The listing builds one solid part. Answer for the finished solid, in the listing's coordinates (mm). Face numbers are marked on the shaded views. A direction names the side the tool comes from. Coordinates: 2 decimals unless noted, no trailing zeros. Order: outer loops, then holes, each group sorted by start corner. A loop starts at its lowest first (then second) coordinate and runs counter-clockwise, first axis right, second up. Notation, with made-up numbers: (87, 60.5) - (143, 60.5) arc R20 cw to (143, 82.5) - close; hole circle Ø10 at (-11, 73). An arc over 180 degrees is marked (long way). Use a Markdown table: item, result. Add a question column.
Item 1: For the marked faces 1, 2 and 3, determine the directions among +Z, -Z, +X, -X, +Y, -Y from which every point of the face is accessible in a straight line to the end or side of a thin tool.
Item 2: The part is cut by section B-B, the plane x = 10. Give the vertices of the cut face in (y, z), then the cut area to 3 significant figures.
Item 3: Find the intervals of material crossed by line 1 along X through (y, z) = (2.25, 5.5); line 2 along Z through (x, y) = (-37, 0.5); line 3 along Z through (x, y) = (-64.5, 0.5), in increasing order.
Item 4: The part is cut by section C-C, the plane x = -9. Give the vertices of the cut face in (y, z).
Item 5: Flat-ended cylindrical pins translate along their axes: P1, Ø3, axis at x = -31.5, z = -3, coming from the +Y side; P2, Ø0.7, axis at x = -36, y = 6.5, coming from the -Z side; P3, Ø2, axis at x = 11, y = 5, coming from the -Z side. Find the tip coordinate at first contact, or state that the pin passes through.
Item 6: The part is cut by section D-D, the plane x = -23. Give the vertices of the cut face in (y, z), then the cut area to 3 significant figures.
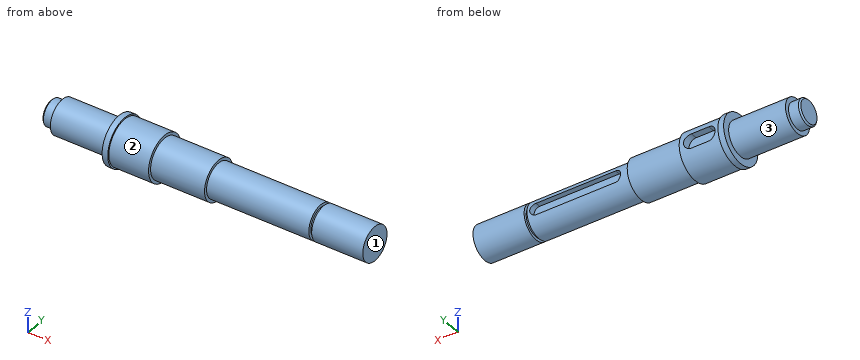
from build123d import *

# Parameters (mm, degrees)
CUT_EXTRUDE_1_DEPTH = 2.2
CUT_EXTRUDE_2_DEPTH = 2.8


with BuildPart() as part:
    # 草图1 → 旋转1 (revolve)
    with BuildSketch(Plane.XY, mode=Mode.PRIVATE) as revolve_1_sk:
        Polygon((-46.103902345, 8.5), (-44.103902345, 8.5), (-44.103902345, 8), (-30.103902345, 8), (-30.103902345, 7), (-11.103902345, 7), (-11.103902345, 6), (24.896097655, 6), (24.896097655, 5), (25.896097655, 5), (25.896097655, 6), (43.896097655, 6), (43.896097655, 0), (-70.103902345, 0), (-70.103902345, 4), (-69.603902345, 4.5), (-66.103902345, 4.5), (-66.103902345, 6), (-46.103902345, 6), align=None)
    revolve(revolve_1_sk.sketch.rotate(Axis((-70.103902345, 0, 0), (1, 0, 0)), 90), axis=Axis((-70.103902345, 0, 0), (1, 0, 0)))

    # 草图7 → 切除-拉伸1 (cut)
    with BuildSketch(Plane(origin=(0, 6, 0), x_dir=(1, 0, 0), z_dir=(0, 1, 0))):
        with BuildLine():
            Line((-6.053902345, 2), (21.946097655, 2))
            ThreePointArc((21.946097655, 2), (23.946097655, 0), (21.946097655, -2))
            Line((21.946097655, -2), (-6.053902345, -2))
            ThreePointArc((-6.053902345, -2), (-8.053902345, 0), (-6.053902345, 2))
        make_face()
    extrude(amount=-CUT_EXTRUDE_1_DEPTH, mode=Mode.SUBTRACT)

    # 草图9 → 切除-拉伸2 (cut)
    with BuildSketch(Plane(origin=(0, 8, 0), x_dir=(1, 0, 0), z_dir=(0, 1, 0))):
        with BuildLine():
            Line((-40.225350305, 2.5), (-34.103902345, 2.5))
            ThreePointArc((-34.103902345, 2.5), (-31.603902345, 0), (-34.103902345, -2.5))
            Line((-34.103902345, -2.5), (-40.225350305, -2.5))
            ThreePointArc((-40.225350305, -2.5), (-42.725350305, 0), (-40.225350305, 2.5))
        make_face()
    extrude(amount=-CUT_EXTRUDE_2_DEPTH, mode=Mode.SUBTRACT)


solid = part.part
Solution:
| question | item | result |
|---|---|---|
| 1 | face 1 | +Z, -Z, +X, +Y, -Y |
| 1 | face 2 | +X |
| 1 | face 3 | -X |
| 2 | outline | (3.8, -2) - (3.8, 2) - (5.66, 2) arc R6 ccw (long way) to (5.66, -2) - close |
| 2 | area | 105 mm2 |
| 3 | line 1 | x = -66.1 to 24.9, 25.9 to 43.9 |
| 3 | line 2 | z = -7.98 to 7.98 |
| 3 | line 3 | z = -5.98 to 5.98 |
| 4 | outline | circle Ø12 at (0, 0) |
| 5 | P1 | stops at y = 7.86 |
| 5 | P2 | stops at z = -5.12 |
| 5 | P3 | stops at z = -4.47 |
| 6 | outline | circle Ø14 at (0, 0) |
| 6 | area | 154 mm2 |
